Work out the finished part from the listing and answer in its coordinate system (mm). Give positions to 0.01 mm unless a question says otherwise; leave off trailing zeros. Loops run counter-clockwise (first coordinate to the right, second up) from the corner with the lowest first, then second, coordinate; pieces in that order, holes last.
```python
from build123d import *

# Parameters (mm, degrees)
SKETCH1_R             = 5
BOSS_EXTRUDE1_DEPTH   = 100
M3_TAPPED_HOLE1_D     = 2.5
M3_TAPPED_HOLE1_DEPTH = 6.5
M3_TAPPED_HOLE1_TIP   = 0.751075774
CHAMFER1_SIZE         = 1
CHAMFER2_SIZE         = 0.5


with BuildPart() as part:
    # Sketch1 → Boss-Extrude1 (new body)
    with BuildSketch(Plane.XY):
        Circle(SKETCH1_R)
    extrude(amount=BOSS_EXTRUDE1_DEPTH)

    # M3 Tapped Hole1
    with Locations(Plane.XY.offset(100)):
        with Locations((0, 0)):
            Hole(M3_TAPPED_HOLE1_D / 2, depth=M3_TAPPED_HOLE1_DEPTH)
            with Locations((0, 0, -(M3_TAPPED_HOLE1_DEPTH + M3_TAPPED_HOLE1_TIP / 2))):  # 118° drill point
                Cone(0, M3_TAPPED_HOLE1_D / 2, M3_TAPPED_HOLE1_TIP, mode=Mode.SUBTRACT)

    # Chamfer1
    chamfer1_edges = [part.edges().sort_by_distance(p)[0] for p in [
        (-5, 0, 0),
        (-5, 0, 100),
    ]]
    chamfer(chamfer1_edges, length=CHAMFER1_SIZE)

    # Chamfer2
    chamfer2_edges = [part.edges().sort_by_distance(p)[0] for p in [
        (1.25, 0, 100),
    ]]
    chamfer(chamfer2_edges, length=CHAMFER2_SIZE)


solid = part.part
```
Q1. Section A-A on z = 29 is taken. Give the vertices of the cut face in (x, y).
Q2. Given pin 1 (1 mm diameter, centred on x = 3, z = 43, fed in from -Y); pin 2 (2 mm diameter, centred on y = 3, z = 43.5, fed in from -X); pin 3 (2 mm diameter, centred on y = 3, z = 74, fed in from +X), each flat-ended and moving along its own axis, determine where each tip first touches the part or whether it passes through.
Q3. Consider line 1 along Y through (x, z) = (0, 95.5); line 2 along Y through (x, z) = (-0.25, 54.5); line 3 along X through (y, z) = (-3, 68). Determine where each line is inside the solid, lowest interval first.
Q4. Determine the mould class of faces 1 (the face through (0.27, -1.22, 96.46)), 2 (the face through (-1.08, -4.88, 49.31)), 3 (the face through (0, 0, 0)) for opening direction X: +X half, -X half, draft (parallel to the pull), parting line (faces both ways), or undercut.
Check result:
1. outline: circle Ø10 at (0, 0)
2. pin 1: stops at y = -4.33
2. pin 2: stops at x = -4.58
2. pin 3: stops at x = 4.58
3. line 1: y = -5 to -1.25, 1.25 to 5
3. line 2: y = -4.99 to 4.99
3. line 3: x = -4 to 4
4. face 1: undercut
4. face 2: parting line
4. face 3: draft
